Check sheet for the modelled part. Datum: model origin and axes. Units: mm. A direction names the side the tool comes from. Round coordinates to 2 decimals unless told otherwise and drop trailing zeros. Write each loop counter-clockwise with the first axis right and the second up, starting at its lowest first coordinate (ties: lowest second). Pieces come first, ordered by that corner, then holes. Notation, with made-up numbers: (56, 14.5) -> (77, 14.5) arc R16 ccw to (77, 24.5) -> close; hole circle Ø6 at (-26, 18). An arc over 180 degrees is marked (long way). One line per item, written item: value.
from build123d import *

# Parameters (mm, degrees)
LEVER_ARM_PROFILE_SKETCH_R = 5
LEVER_ARM_BODY_DEPTH       = 60
ARM_RELIEF_CUT_DEPTH       = 112.018016556
ARM_RELIEF_CUT_DEPTH_BACK  = 112.018016556


with BuildPart() as part:
    # Lever Arm Profile Sketch → Lever Arm Body (new body)
    with BuildSketch(Plane.XY):
        with BuildLine():
            Line((81.822654266, 9.832493652), (4.687544359, 24.556606604))
            ThreePointArc((4.687544359, 24.556606604), (-25, 0), (4.687544359, -24.556606604))
            Line((4.687544359, -24.556606604), (81.822654266, -9.832493652))
            ThreePointArc((81.822654266, -9.832493652), (90, 0), (81.822654266, 9.832493652))
        make_face()
        with Locations(Location((80, 0, 0), (0, 0, 180))):
            Circle(LEVER_ARM_PROFILE_SKETCH_R, mode=Mode.SUBTRACT)
        with BuildLine():
            Line((60.79258109, 7.5), (27.739398554, 11.641553498))
            ThreePointArc((27.739398554, 11.641553498), (24.632664937, 10.429819806), (23.951098456, 7.165534365))
            ThreePointArc((23.951098456, 7.165534365), (25, 0), (23.951098456, -7.165534365))
            ThreePointArc((23.951098456, -7.165534365), (24.632664937, -10.429819806), (27.739398554, -11.641553498))
            Line((27.739398554, -11.641553498), (60.79258109, -7.5))
            ThreePointArc((60.79258109, -7.5), (68.29258109, 0), (60.79258109, 7.5))
        make_face(mode=Mode.SUBTRACT)
        with BuildLine():
            Line((10, 17.071067812), (6.464466094, 13.535533906))
            ThreePointArc((6.464466094, 13.535533906), (-10.606601718, -10.606601718), (13.535533906, 6.464466094))
            Line((13.535533906, 6.464466094), (17.071067812, 10))
            Line((17.071067812, 10), (10, 17.071067812))
        make_face(mode=Mode.SUBTRACT)
    extrude(amount=LEVER_ARM_BODY_DEPTH)

    # Relief Cut Profile Sketch → Arm Relief Cut (cut, two sides: drawn at the far end of the back side and taken through both)
    with BuildSketch(Plane(origin=(0, 0, 0), x_dir=(1, 0, 0), z_dir=(0, 1, 0)).offset(-ARM_RELIEF_CUT_DEPTH_BACK)):
        with BuildLine():
            Line((18.654539923, -14), (-25, -14))
            Line((-25, -14), (-25, -60))
            Line((-25, -60), (70.709652312, -60))
            ThreePointArc((70.709652312, -60), (61.268398012, -57.631299364), (54.063494219, -51.086271725))
            Line((54.063494219, -51.086271725), (35.300698016, -22.913728275))
            ThreePointArc((35.300698016, -22.913728275), (28.095794223, -16.368700636), (18.654539923, -14))
        make_face()
        with BuildLine():
            Line((53.654787377, -8), (90, -8))
            Line((90, -8), (90, -52))
            Line((90, -52), (69.638687081, -52))
            ThreePointArc((69.638687081, -52), (64.918059931, -50.815649682), (61.315608035, -47.543135862))
            Line((61.315608035, -47.543135862), (45.331708331, -23.543135862))
            ThreePointArc((45.331708331, -23.543135862), (44.839137696, -13.27937285), (53.654787377, -8))
        make_face()
    extrude(amount=ARM_RELIEF_CUT_DEPTH + ARM_RELIEF_CUT_DEPTH_BACK, mode=Mode.SUBTRACT)


solid = part.part
Item 1: Mould release check, pull along Z, two halves, no side actions. Record for faces 4 (the flat face through (44.813, -13.601, 37.197)), 5 (the cylindrical face through (44.77, 12.75, 13.41)), 6 (the cylindrical face through (-24.992, 0.616, 6.902)): pulls with the +Z half, pulls with the -Z half, needs draft (parallel to the pull), parting line crosses it, or undercut.
Answer:
face 4: pulls with the +Z half
face 5: undercut
face 6: needs draft
Item 2: Depth check by flat-ended pin: P1, Ø18, axis at x = 0, y = 0, coming from the +Z side; P2, Ø13, axis at x = 5.5, y = -8.5, coming from the +Z side; P3, Ø16.5, axis at x = 85, y = 3, coming from the -Z side; P4, Ø1.5, axis at y = -10.5, z = 21, coming from the +X side. Enter the tip coordinate at first touch or a pass-through.
Answer:
P1: passes through
P2: stops at z = 14
P3: stops at z = 0
P4: stops at x = 44.38
Item 3: Sectioned sample at A-A on x = 0. Enter the section's corners in (y, z).
Answer:
outline: (-25, 0) -> (-15, 0) -> (-15, 14) -> (-25, 14) -> close; (15, 0) -> (25, 0) -> (25, 14) -> (15, 14) -> close
Item 4: Sectioned sample at B-B on z = 33. Enter the section's corners in (x, y).
Answer:
outline: (42.02, -17.43) -> (51.63, -15.6) -> (51.63, -8.65) -> (42.02, -9.85) -> close; (42.02, 9.85) -> (51.63, 8.65) -> (51.63, 15.6) -> (42.02, 17.43) -> close
Item 5: Sectioned sample at D-D on x = 80. Enter the section's corners in (y, z), and give its area (3 significant figures).
Answer:
outline: (-10.18, 0) -> (-5, 0) -> (-5, 8) -> (-10.18, 8) -> close; (-10.18, 52) -> (-5, 52) -> (-5, 60) -> (-10.18, 60) -> close; (5, 0) -> (10.18, 0) -> (10.18, 8) -> (5, 8) -> close; (5, 52) -> (10.18, 52) -> (10.18, 60) -> (5, 60) -> close
area: 166 mm^2
Item 6: Sectioned sample at C-C on y = 0. Enter the section's corners in (x, z), and give its area (3 significant figures).
Answer:
outline: (-25, 0) -> (-15, 0) -> (-15, 14) -> (-25, 14) -> close; (15, 0) -> (25, 0) -> (25, 15.03) arc R20 cw to (18.65, 14) -> (15, 14) -> close; (68.29, 0) -> (75, 0) -> (75, 8) -> (68.29, 8) -> close; (68.29, 51.91) arc R10 cw to (69.64, 52) -> (75, 52) -> (75, 60) -> (70.71, 60) arc R20 ccw to (68.29, 59.85) -> close; (85, 0) -> (90, 0) -> (90, 8) -> (85, 8) -> close; (85, 52) -> (90, 52) -> (90, 60) -> (85, 60) -> close
area: 469 mm^2
Item 7: Thickness scan on line 1 (Z direction, x = -15, y = 13); line 2 (Y direction, x = 34, z = 14.5); line 3 (X direction, y = -2.5, z = 56). Record the ranges inside material, lowest first.
Answer:
line 1: z = 0 to 14
line 2: y = -18.96 to -10.86, 10.86 to 18.96
line 3: x = 67.86 to 75.67, 84.33 to 89.68
Item 8: Tool access check on faces 1 (the flat face through (-13, 11, 14)), 2 (the flat face through (13.585, 13.486, 6.902)), 3 (the flat face through (72, 0, 8)). Record the directions out of +Z, -Z, +X, -X, +Y, -Y that give a thin tool (end or side, any length) a straight path to the whole face; none if there is none.
Answer:
face 1: +Z, -X, +Y, -Y
face 2: +Z, -Z
face 3: +X, +Y, -Y
